Can you work these out from the model? Positions are in its coordinate system, mm. A direction names the side the tool comes from. Give positions to 0.01 mm unless a question says otherwise; leave off trailing zeros. Order: outer loops, then holes, each group sorted by start corner. A loop starts at its lowest first (then second) coordinate and runs counter-clockwise, first axis right, second up. Notation, with made-up numbers: (71.25, 16.5) - (119.25, 16.5) arc R22 ccw to (119.25, 47.5) - close; hole circle Ø7 at (24, 38). An arc over 180 degrees is marked (long way). Answer as a JSON object with one key per item and string values.
```python
from build123d import *

# Parameters (mm, degrees)
SKETCH1_W           = 25
SKETCH1_H           = 62
BOSS_EXTRUDE1_DEPTH = 7
SKETCH2_R           = 5
BOSS_EXTRUDE2_DEPTH = 56
SKETCH3_R           = 5
BOSS_EXTRUDE3_DEPTH = 56
HOLE1_D             = 3
HOLE1_DEPTH         = 6
HOLE1_TIP           = 0.866025404
CUT_EXTRUDE1_DEPTH  = 3
HOLE2_D             = 3
HOLE2_DEPTH         = 6
HOLE2_TIP           = 0.866025404
SKETCH14_W          = 10
SKETCH14_H          = 56
CUT_EXTRUDE2_DEPTH  = 4.5


with BuildPart() as part:
    # Sketch1 → Boss-Extrude1 (new body)
    with BuildSketch(Plane.XY.offset(13)):
        Rectangle(SKETCH1_W, SKETCH1_H)
    extrude(amount=-BOSS_EXTRUDE1_DEPTH)

    # Sketch2 → Boss-Extrude2 (add)
    with BuildSketch(Plane.XY.offset(13)):
        with Locations((0, 23)):
            Circle(SKETCH2_R)
    extrude(amount=-BOSS_EXTRUDE2_DEPTH)

    # Sketch3 → Boss-Extrude3 (add)
    with BuildSketch(Plane.XY.offset(13)):
        with Locations((0, -23)):
            Circle(SKETCH3_R)
    extrude(amount=-BOSS_EXTRUDE3_DEPTH)

    # Sketch4 → Revolve1 (revolve)
    with BuildSketch(Plane(origin=(0, 0, 0), x_dir=(0, 0, -1), z_dir=(1, 0, 0)), mode=Mode.PRIVATE) as revolve1_sk:
        Polygon((-6, 0), (-6, 4), (20.5, 4), (20.5, 8), (25.5, 8), (25.5, 0), align=None)
    revolve(revolve1_sk.sketch.rotate(Axis((0, 0, -25.5), (0, 0, 1)), 270), axis=Axis((0, 0, -25.5), (0, 0, 1)))

    # Hole1
    with Locations(Plane.XY.offset(13)):
        with Locations((0, 12)):
            Hole(HOLE1_D / 2, depth=HOLE1_DEPTH)
            with Locations((0, 0, -(HOLE1_DEPTH + HOLE1_TIP / 2))):  # 120° drill point
                Cone(0, HOLE1_D / 2, HOLE1_TIP, mode=Mode.SUBTRACT)

    # Sketch7 → Cut-Extrude1 (cut)
    with BuildSketch(Plane.XY.offset(13)):
        with BuildLine():
            Line((1.5, 11.75), (1.5, 12.25))
            ThreePointArc((1.5, 12.25), (0, 13.75), (-1.5, 12.25))
            Line((-1.5, 12.25), (-1.5, 11.75))
            ThreePointArc((-1.5, 11.75), (0, 10.25), (1.5, 11.75))
        make_face()
    extrude(amount=-CUT_EXTRUDE1_DEPTH, mode=Mode.SUBTRACT)

    # Hole2
    with Locations(Plane.XY.offset(13)):
        with Locations((0, -12)):
            Hole(HOLE2_D / 2, depth=HOLE2_DEPTH)
            with Locations((0, 0, -(HOLE2_DEPTH + HOLE2_TIP / 2))):  # 120° drill point
                Cone(0, HOLE2_D / 2, HOLE2_TIP, mode=Mode.SUBTRACT)

    # Sketch10 → Cut-Revolve1 (revolve, cut)
    with BuildSketch(Plane(origin=(0, -27, 0), x_dir=(1, 0, 0), z_dir=(0, 1, 0)), mode=Mode.PRIVATE) as cut_revolve1_sk:
        Polygon((8, -6), (10.5, -6), (10.067, -6.433), (10.067, -12.567), (10.5, -13), (8, -13), align=None)
    revolve(cut_revolve1_sk.sketch.rotate(Axis((8, -27, 13), (0, 0, -1)), 180), axis=Axis((8, -27, 13), (0, 0, -1)), mode=Mode.SUBTRACT)

    # Sketch11 → Cut-Revolve2 (revolve, cut)
    with BuildSketch(Plane(origin=(0, -27, 0), x_dir=(1, 0, 0), z_dir=(0, 1, 0)), mode=Mode.PRIVATE) as cut_revolve2_sk:
        Polygon((-8, -6), (-5.5, -6), (-5.933, -6.433), (-5.933, -12.567), (-5.5, -13), (-8, -13), align=None)
    revolve(cut_revolve2_sk.sketch.rotate(Axis((-8, -27, 13), (0, 0, -1)), 180), axis=Axis((-8, -27, 13), (0, 0, -1)), mode=Mode.SUBTRACT)

    # Sketch12 → Cut-Revolve3 (revolve, cut)
    with BuildSketch(Plane(origin=(0, 27, 0), x_dir=(1, 0, 0), z_dir=(0, 1, 0)), mode=Mode.PRIVATE) as cut_revolve3_sk:
        Polygon((8, -6), (10.5, -6), (10.067, -6.433), (10.067, -12.567), (10.5, -13), (8, -13), align=None)
    revolve(cut_revolve3_sk.sketch.rotate(Axis((8, 27, 13), (0, 0, -1)), 180), axis=Axis((8, 27, 13), (0, 0, -1)), mode=Mode.SUBTRACT)

    # Sketch13 → Cut-Revolve4 (revolve, cut)
    with BuildSketch(Plane(origin=(0, 27, 0), x_dir=(1, 0, 0), z_dir=(0, 1, 0)), mode=Mode.PRIVATE) as cut_revolve4_sk:
        Polygon((-8, -6), (-5.5, -6), (-5.933, -6.433), (-5.933, -12.567), (-5.5, -13), (-8, -13), align=None)
    revolve(cut_revolve4_sk.sketch.rotate(Axis((-8, 27, 13), (0, 0, -1)), 180), axis=Axis((-8, 27, 13), (0, 0, -1)), mode=Mode.SUBTRACT)

    # Sketch14 → Cut-Extrude2 (cut)
    with BuildSketch(Plane(origin=(0, 0, -43), x_dir=(-1, 0, 0), z_dir=(0, 0, -1))):
        Rectangle(SKETCH14_W, SKETCH14_H)
    extrude(amount=-CUT_EXTRUDE2_DEPTH, mode=Mode.SUBTRACT)


solid = part.part
```
Q1. I need wall thicknesses on L1, parallel to Y at x = -8, z = 9.75; L2, parallel to Y at x = 0, z = 8.25; L3, parallel to Z at x = 5.25, y = 3.5. Which ranges of each line are inside material? Lowest first, please.
Recorded:
{"L1": "y = -31 to -29.07, -24.93 to 24.93, 29.07 to 31", "L2": "y = -31 to -13.5, -10.5 to 10.5, 13.5 to 31", "L3": "z = -25.5 to -20.5, 6 to 13"}
Q2. I'm going to push flat-ended pins straight in: pin 1 Ø1.8 at (x, y) = (0, 12) entering from -Z; pin 2 Ø3.5 at (x, y) = (8, -27) entering from -Z; pin 3 Ø0.9 at (x, y) = (0, 12.5) entering from +Z; pin 4 Ø10 at (x, y) = (-1, 11.5) entering from -Z. Where does each tip first touch, or does it pass through?
Recorded:
{"pin 1": "stops at z = 6", "pin 2": "passes through", "pin 3": "stops at z = 6.68", "pin 4": "stops at z = -25.5"}
Q3. If we section it at D-D, the plane y = 23: Please give me the cut outline in (x, z), then the cut area to 3 significant figures.
Recorded:
{"outline": "(-12.5, 6) - (-5, 6) - (-5, -38.5) - (5, -38.5) - (5, 6) - (12.5, 6) - (12.5, 13) - (-12.5, 13) - close", "area": "620 mm^2"}
Q4. Which directions (+Z, -Z, +X, -X, +Y, -Y) give clear straight access to the entire face, cutting with the end or side of a thin tool? Please do faces 5 (the face through (-1.08, -27.88, -15.94)), 6 (the face through (12.5, 0, 10)), 7 (the face through (0.03, 13.75, 11.52)).
Recorded:
{"face 5": "-Z", "face 6": "+Z, -Z, +X, +Y, -Y", "face 7": "+Z"}
Q5. If we section it at C-C, the plane z = -34.5: Please give me the cut outline in (x, y).
Recorded:
{"outline": "circle Ø10 at (0, -23); circle Ø10 at (0, 23)"}
Q6. If we section it at A-A, the plane y = -27: Please give me the cut outline in (x, z).
Recorded:
{"outline": "(-12.5, 6) - (-10.5, 6) - (-10.07, 6.43) - (-10.07, 12.57) - (-10.5, 13) - (-12.5, 13) - close; (-5.93, 6.43) - (-5.5, 6) - (-3, 6) - (-3, -38.5) - (3, -38.5) - (3, 6) - (5.5, 6) - (5.93, 6.43) - (5.93, 12.57) - (5.5, 13) - (-5.5, 13) - (-5.93, 12.57) - close; (10.07, 6.43) - (10.5, 6) - (12.5, 6) - (12.5, 13) - (10.5, 13) - (10.07, 12.57) - close"}
Q7. If we section it at B-B, the plane x = -2.5: Please give me the cut outline in (y, z).
Recorded:
{"outline": "(-31, 6) - (-27.33, 6) - (-27.33, -38.5) - (-18.67, -38.5) - (-18.67, 6) - (-3.12, 6) - (-3.12, -20.5) - (-7.6, -20.5) - (-7.6, -25.5) - (7.6, -25.5) - (7.6, -20.5) - (3.12, -20.5) - (3.12, 6) - (18.67, 6) - (18.67, -38.5) - (27.33, -38.5) - (27.33, 6) - (31, 6) - (31, 13) - (-31, 13) - close"}
Q8. We'd pull the mould along X, two halves only. Please class faces 1 (the face through (0, 0, 13)), 2 (the face through (-12.5, 0, 10)), 3 (the face through (-7.552, 24.982, 9.543)), 4 (the face through (0.12, -12.231, 6.284)): released by +X, released by -X, zero draft, split by the parting line, or undercut.
Recorded:
{"face 1": "zero draft", "face 2": "released by -X", "face 3": "undercut", "face 4": "undercut"}
